Could you check a few things on this model? Use its own coordinates, in mm. Give positions to 0.01 mm unless a question says otherwise; leave off trailing zeros. Order: outer loops, then holes, each group sorted by start corner. A loop starts at its lowest first (then second) coordinate and runs counter-clockwise, first axis right, second up.
from build123d import *

# Parameters (mm, degrees)
BASEKEY_DEPTH = 3.5
CHAMFER1_SIZE = 0.4


with BuildPart() as part:
    # Sketch1 → BaseKey (new, symmetric)
    with BuildSketch(Plane.XY):
        with BuildLine():
            Line((-12, 4), (0, 4))
            ThreePointArc((0, 4), (4, 0), (0, -4))
            Line((0, -4), (-12, -4))
            ThreePointArc((-12, -4), (-16, 0), (-12, 4))
        make_face()
    extrude(amount=BASEKEY_DEPTH, both=True)

    # Chamfer1
    chamfer1_edges = [part.edges().sort_by_distance(p)[0] for p in [
        (4, 0, 3.5),
        (-6, 4, 3.5),
        (-16, 0, 3.5),
        (-6, 4, -3.5),
        (4, 0, -3.5),
        (-6, -4, -3.5),
        (-16, 0, -3.5),
        (-6, -4, 3.5),
    ]]
    chamfer(chamfer1_edges, length=CHAMFER1_SIZE)


solid = part.part
Item 1: Please list where these lines run through material, in increasing order: line 1 along X through (y, z) = (1.75, -0.5); line 2 along X through (y, z) = (-0.5, 0.75); line 3 along Y through (x, z) = (1, -1).
Findings:
line 1: x = -15.6 to 3.6
line 2: x = -15.97 to 3.97
line 3: y = -3.87 to 3.87
Item 2: Imagine slicing it at A-A on z = 1. List the corners of the cut face in (x, y) for me.
Findings:
outline: (-12, -4) - (0, -4) arc R4 ccw to (0, 4) - (-12, 4) arc R4 ccw to start
Item 3: For pin 1 (3 mm diameter, centred on y = -1, z = 0, fed in from +X), with a flat end and sliding along its axis, tell me the tip position at first contact or that it passes through.
Findings:
pin 1: stops at x = 4
